from build123d import *

# Parameters (mm, degrees)
CUT_EXTRUDE_START   = -2e-06
SKETCH_3_OUTSIDE_W  = 78.998
SKETCH_3_OUTSIDE_H  = 78.998
CUT_EXTRUDE_2_DEPTH = 4.764157
SKETCH_4_W          = 5.7
SKETCH_4_H          = 1.5
EXTRUDE_1_DEPTH     = 5


with BuildPart() as part:
    # 草图2 → Revolve 544 (revolve)
    with BuildSketch(Plane(origin=(0, 0, 0), x_dir=(0, 0, -1), z_dir=(1, 0, 0))):
        Polygon((-3.264153607, 30), (0, 23), (0, 0), (-1.5, 0), (-1.5, 23), (-4.764153607, 30), align=None)
    revolve(axis=Axis((0, 0, 0), (0, 0, 1)))

    # 草图3 outside → 切除-拉伸2 (cut)
    # profile 1 of 2: a face of its own
    with BuildSketch(Plane.XY.offset(CUT_EXTRUDE_START)):
        Rectangle(SKETCH_3_OUTSIDE_W, SKETCH_3_OUTSIDE_H)
        with BuildLine():
            Line((-2.85, -22.822740852), (-2.85, -29.864318174))
            Line((-2.85, -29.864318174), (2.85, -29.864318174))
            Line((2.85, -29.864318174), (2.85, -22.822740852))
            ThreePointArc((2.85, -22.822740852), (18.247126827, -14.001512867), (22.782709094, 3.154071389))
            Line((22.782709094, 3.154071389), (29.584350487, 4.976565708))
            Line((29.584350487, 4.976565708), (28.10908193, 10.482342917))
            Line((28.10908193, 10.482342917), (21.307440537, 8.659848599))
            ThreePointArc((21.307440537, 8.659848599), (19.918584287, 11.5), (18.153369148, 14.122860495))
            Line((18.153369148, 14.122860495), (23.132516223, 19.10200757))
            Line((23.132516223, 19.10200757), (19.10200757, 23.132516223))
            Line((19.10200757, 23.132516223), (14.122860495, 18.153369148))
            ThreePointArc((14.122860495, 18.153369148), (11.5, 19.918584287), (8.659848599, 21.307440537))
            Line((8.659848599, 21.307440537), (10.482342917, 28.10908193))
            Line((10.482342917, 28.10908193), (4.976565708, 29.584350487))
            Line((4.976565708, 29.584350487), (3.154071389, 22.782709094))
            ThreePointArc((3.154071389, 22.782709094), (-18.247126827, 14.001512867), (-21.190073362, -8.943198025))
            Line((-21.190073362, -8.943198025), (-27.288258205, -12.463986686))
            Line((-27.288258205, -12.463986686), (-24.438258205, -17.400331488))
            Line((-24.438258205, -17.400331488), (-18.340073362, -13.879542827))
            ThreePointArc((-18.340073362, -13.879542827), (-16.263455967, -16.263455967), (-13.879542827, -18.340073362))
            Line((-13.879542827, -18.340073362), (-17.400331488, -24.438258205))
            Line((-17.400331488, -24.438258205), (-12.463986686, -27.288258205))
            Line((-12.463986686, -27.288258205), (-8.943198025, -21.190073362))
            ThreePointArc((-8.943198025, -21.190073362), (-5.952838037, -22.216294005), (-2.85, -22.822740852))
        make_face(mode=Mode.SUBTRACT)
    # profile 2 of 2: a face of its own
    with BuildSketch(Plane.XY.offset(CUT_EXTRUDE_START)):
        with BuildLine():
            Line((2.85, -18.0260922), (2.85, -14.75))
            Line((2.85, -14.75), (-2.85, -14.75))
            Line((-2.85, -14.75), (-2.85, -18.0260922))
            ThreePointArc((-2.85, -18.0260922), (0, 18.25), (2.85, -18.0260922))
        make_face()
    extrude(amount=CUT_EXTRUDE_2_DEPTH, mode=Mode.SUBTRACT)

    # 草图4 → 凸台-拉伸1 (add)
    with BuildSketch(Plane.XY):
        with Locations((0, -15.5)):
            Rectangle(SKETCH_4_W, SKETCH_4_H)
    extrude(amount=EXTRUDE_1_DEPTH)


solid = part.part
Geometry check sheet. Reference: the model listing, model coordinates, mm. A direction names the side the tool comes from. Give positions to 0.01 mm unless a question says otherwise; leave off trailing zeros. Order: outer loops, then holes, each group sorted by start corner. A loop starts at its lowest first (then second) coordinate and runs counter-clockwise, first axis right, second up.
1) Draft check along Y on faces 4 (the flat face through (-2.85, -16, 2)), 5 (the flat face through (0, -15, 0)), 6 (the conical face through (18.74, 18.67, 1.61)). Enter one of: released by +Y, released by -Y, zero draft, split by the parting line, or undercut.
Results are:
face 4: undercut
face 5: zero draft
face 6: released by +Y
2) Cross-section at C-C (x = 0). Record the boundary of the cut face in (y, z).
Results are:
outline: (-29.86, 3.2) - (-23, 0) - (-14.75, 0) - (-14.75, 5) - (-16.25, 5) - (-16.25, 1.5) - (-23, 1.5) - (-29.86, 4.7) - close; (18.25, 0) - (23, 0) - (23, 1.5) - (18.25, 1.5) - close
3) Gauge pin test, flat ends, axial feed: pin 1 (1 mm diameter, centred on y = 7, z = 3.5, fed in from -X); pin 2 (1.5 mm diameter, centred on x = -0.5, z = 3, fed in from +Y); pin 3 (1 mm diameter, centred on y = -16, z = 3, fed in from -X). Record the tip position at first contact, or that the pin passes through.
Results are:
pin 1: stops at x = 25.26
pin 2: stops at y = -14.75
pin 3: stops at x = -25.51
4) Cross-section at A-A (y = 0). Record the boundary of the cut face in (x, z).
Results are:
outline: (-23, 0) - (-18.25, 0) - (-18.25, 1.5) - (-23, 1.5) - close; (18.25, 0) - (23, 0) - (23, 1.5) - (18.25, 1.5) - close
5) Material ranges on probe 1 along X at (y, z) = (0, 1); probe 2 along X at (y, z) = (9.5, 1.15); probe 3 along Z at (x, y) = (-20, 1), recorded low to high.
Results are:
probe 1: x = -23 to -18.25, 18.25 to 23
probe 2: x = -20.95 to -15.58, 15.58 to 20.95
probe 3: z = 0 to 1.5
6) Cross-section at B-B (z = 2.4). Record the boundary of the cut face in (x, y), then the cut area to 3 significant figures.
Results are:
outline: (-25.68, -11.53) arc R28.15 ccw to (-22.83, -16.47) - (-20.02, -14.85) arc R24.93 cw to (-22.87, -9.92) - close; (-16.47, -22.83) arc R28.15 ccw to (-11.53, -25.68) - (-9.92, -22.87) arc R24.93 cw to (-14.85, -20.02) - close; (-2.85, -28) arc R28.15 ccw to (2.85, -28) - (2.85, -24.77) arc R24.93 cw to (-2.85, -24.77) - close; (-2.85, -16.25) - (2.85, -16.25) - (2.85, -14.75) - (-2.85, -14.75) - close; (3.66, 24.66) arc R24.93 cw to (9.16, 23.19) - (10, 26.31) arc R28.15 ccw to (4.49, 27.79) - close; (15.5, 19.53) arc R24.93 cw to (19.53, 15.5) - (21.82, 17.79) arc R28.15 ccw to (17.79, 21.82) - close; (23.19, 9.16) arc R24.93 cw to (24.66, 3.66) - (27.79, 4.49) arc R28.15 ccw to (26.31, 10) - close
area: 119 mm2
7) Tool access check on faces 1 (the flat face through (2.85, -26, 2)), 2 (the flat face through (0, -16.25, 3)), 3 (the cylindrical face through (-16.295, -16.232, 0.74)). Record the directions out of +Z, -Z, +X, -X, +Y, -Y that give a thin tool (end or side, any length) a straight path to the whole face; none if there is none.
Results are:
face 1: +Z, -Z, +X, -Y
face 2: +Z, +X
face 3: +Z, -Z
8) Cross-section at D-D (x = -6). Record the boundary of the cut face in (y, z), then the cut area to 3 significant figures.
Results are:
outline: (-22.2, 0) - (-17.24, 0) - (-17.24, 1.5) - (-22.2, 1.5) - close; (17.24, 0) - (22.2, 0) - (22.2, 1.5) - (17.24, 1.5) - close
area: 14.9 mm2
